The listing builds one solid part. Answer for the finished solid, in the listing's coordinates (mm). Face numbers are marked on the shaded views. A direction names the side the tool comes from. Round coordinates to 2 decimals unless told otherwise and drop trailing zeros. Order: outer loops, then holes, each group sorted by start corner. A loop starts at its lowest first (then second) coordinate and runs counter-clockwise, first axis right, second up. Notation, with made-up numbers: M 46,52 L 89,52 A24 ccw 89,77 Z; hole C 10,-18 d6. An arc over 180 degrees is marked long. Put each result on its own line as item: value. Start each with the question number.
1. The part is cut by section C-C (y = 59.5). Give the vertices of the cut face in (x, z), then the cut area to 3 significant figures.
2. The part is cut by section A-A (z = 10). Count the separate pieces of the cut face and the enclosed holes in it, then the cut area to 3 significant figures.
3. The part is cut by section D-D (z = -8.5). Give the vertices of the cut face in (x, y), then the cut area to 3 significant figures.
4. Each of these flat-tipped pins is pushed along its axis until it touches: pin 1 Ø6 at (x, z) = (0, -4.5) entering from -Y; pin 2 Ø3 at (x, y) = (20.5, 45.5) entering from +Z; pin 3 Ø4 at (y, z) = (50, 13.5) entering from -X. Where does it stop, or does it pass through?
5. Which of the six approach directions +Z, -Z, +X, -X, +Y, -Y give full straight-line access (tool end or side, diameter ignored) to the marked faces 5, 6 and 7?
6. Consider line 1 (X direction, y = 57.75, z = 10); line 2 (Y direction, x = -5, z = -6.5); line 3 (Y direction, x = 6, z = 39.5). Determine where each line is inside the solid, lowest interval first.
7. The mould has two halves that part along Y. Classify the marked faces 1, 2, 3 and 4: +Y half, -Y half, draft (parallel to the pull), parting line (faces both ways), or undercut.
8. The part is cut by section B-B (x = 9). Give the vertices of the cut face in (y, z), then the cut area to 3 significant figures.
from build123d import *

# Parameters (mm, degrees)
BOSS_EXTRUDE4_DEPTH      = 20
BOSS_EXTRUDE5_REACH      = 41.361
BOSS_EXTRUDE5_END_RADIUS = 37.5
SKETCH8_R                = 10
SKETCH9_R                = 20
BOSS_EXTRUDE6_DEPTH      = 5
SKETCH10_R               = 32.5
BOSS_EXTRUDE7_DEPTH      = 20
SKETCH11_R               = 20
BOSS_EXTRUDE8_DEPTH      = 5
SKETCH12_R               = 10
CUT_EXTRUDE3_DEPTH       = 20


with BuildPart() as part:
    # Sketch4 → Boss-Extrude4 (new body)
    with BuildSketch(Plane.XY):
        with BuildLine():
            Line((-26.811555509, 22.497566339), (-28.726666617, 24.104535363))
            ThreePointArc((-28.726666617, 24.104535363), (0, 37.5), (28.726666617, 24.104535363))
            Line((28.726666617, 24.104535363), (26.811555509, 22.497566339))
            ThreePointArc((26.811555509, 22.497566339), (0, 35), (-26.811555509, 22.497566339))
        make_face()
    extrude(amount=BOSS_EXTRUDE4_DEPTH)

    # Boss-Extrude5: up to this cylinder (the profile starts outside it)
    boss_extrude5_end = Plane(origin=(0, 0, 10), z_dir=(0, 0, -1)) * Cylinder(BOSS_EXTRUDE5_END_RADIUS, 158.722, mode=Mode.PRIVATE)
    # Sketch8 → Boss-Extrude5 (add, up to the surface)
    with BuildSketch(Plane(origin=(0, 40.5, 0), x_dir=(1, 0, 0), z_dir=(0, 1, 0)), mode=Mode.PRIVATE) as boss_extrude5_sk1:
        with Locations(Location((0, -10, 0), (0, 0, 270))):
            Circle(SKETCH8_R)
    boss_extrude5_tool1 = extrude(boss_extrude5_sk1.sketch, amount=-BOSS_EXTRUDE5_REACH, mode=Mode.PRIVATE) - boss_extrude5_end
    add(boss_extrude5_tool1.solids().sort_by_distance((0, 40.5, 10))[0])

    # Sketch9 → Boss-Extrude6 (add)
    with BuildSketch(Plane(origin=(0, 40.5, 0), x_dir=(1, 0, 0), z_dir=(0, 1, 0))):
        with Locations(Location((0, -10, 0), (0, 0, 270))):
            Circle(SKETCH9_R)
    extrude(amount=BOSS_EXTRUDE6_DEPTH)

    # Sketch10 → Boss-Extrude7 (add)
    with BuildSketch(Plane(origin=(0, 45.5, 0), x_dir=(1, 0, 0), z_dir=(0, 1, 0))):
        with Locations(Location((0, -10, 0), (0, 0, 270))):
            Circle(SKETCH10_R)
    extrude(amount=BOSS_EXTRUDE7_DEPTH)

    # Sketch11 → Boss-Extrude8 (add)
    with BuildSketch(Plane(origin=(0, 65.5, 0), x_dir=(1, 0, 0), z_dir=(0, 1, 0))):
        with Locations(Location((0, -10, 0), (0, 0, 270))):
            Circle(SKETCH11_R)
    extrude(amount=BOSS_EXTRUDE8_DEPTH)

    # Sketch12 → Cut-Extrude3 (cut)
    with BuildSketch(Plane(origin=(0, 70.5, 0), x_dir=(1, 0, 0), z_dir=(0, 1, 0))):
        with Locations(Location((0, -10, 0), (0, 0, 270))):
            Circle(SKETCH12_R)
    extrude(amount=-CUT_EXTRUDE3_DEPTH, mode=Mode.SUBTRACT)

    # Sketch15 → Cut-Revolve3 (revolve, cut)
    with BuildSketch(Plane.XY.offset(10), mode=Mode.PRIVATE) as cut_revolve3_sk:
        Polygon((-17.693131792, 21.085853377), (-26.278152948, 31.317083182), (-30.108375164, 28.103145134), (-21.523354007, 17.871915328), align=None)
    revolve(cut_revolve3_sk.sketch.rotate(Axis((-17.693131792, 21.085853377, 10), (-0.6427876096865413, 0.7660444431189765, 0)), 180), axis=Axis((-17.693131792, 21.085853377, 10), (-0.6427876096865413, 0.7660444431189765, 0)), mode=Mode.SUBTRACT)

    # Sketch16 → Cut-Revolve4 (revolve, cut)
    with BuildSketch(Plane.XY.offset(10), mode=Mode.PRIVATE) as cut_revolve4_sk:
        Polygon((17.792638641, 21.204441023), (27.637153268, 32.936676696), (23.806931052, 36.150614744), (13.962416426, 24.418379071), align=None)
    revolve(cut_revolve4_sk.sketch.rotate(Axis((17.792638641, 21.204441023, 10), (0.6427876096865399, 0.7660444431189776, 0)), 180), axis=Axis((17.792638641, 21.204441023, 10), (0.6427876096865399, 0.7660444431189776, 0)), mode=Mode.SUBTRACT)


solid = part.part
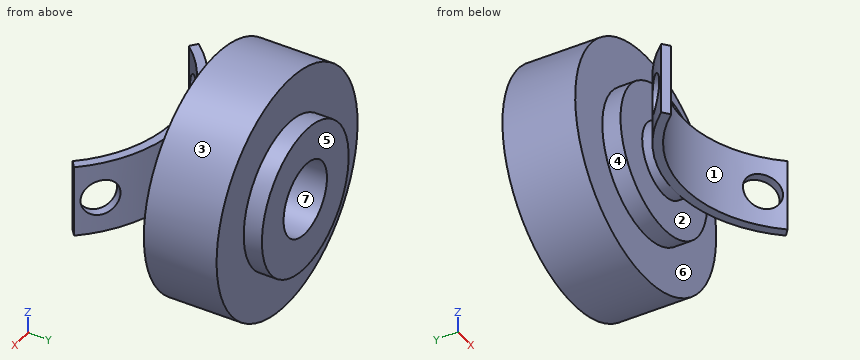
Resolved:
1. outline: C 0,10 d65; hole C 0,10 d20
1. area: 3,000 mm2
2. separate pieces: 3
2. enclosed holes: 0
2. area: 1,480 mm2
3. outline: M -26.72,45.5 L -7.6,45.5 L -7.6,40.5 L 7.6,40.5 L 7.6,45.5 L 26.72,45.5 L 26.72,65.5 L 7.6,65.5 L 7.6,70.5 L -7.6,70.5 L -7.6,65.5 L -26.72,65.5 Z
3. area: 1,220 mm2
4. pin 1: y = 40.5
4. pin 2: z = 36.37
4. pin 3: x = -32.47
5. face 5: +Z, -Z, +X, -X, +Y
5. face 6: none
5. face 7: +Y
6. line 1: -32.5 to -10, 10 to 32.5
6. line 2: 40.5 to 70.5
6. line 3: 45.5 to 65.5
7. face 1: -Y half
7. face 2: undercut
7. face 3: draft
7. face 4: undercut
8. outline: M 33.82,0 L 36.4,0 L 36.4,5.64 L 40.5,5.64 L 40.5,-7.86 L 45.5,-7.86 L 45.5,-21.23 L 65.5,-21.23 L 65.5,-7.86 L 70.5,-7.86 L 70.5,5.64 L 50.5,5.64 L 50.5,14.36 L 70.5,14.36 L 70.5,27.86 L 65.5,27.86 L 65.5,41.23 L 45.5,41.23 L 45.5,27.86 L 40.5,27.86 L 40.5,14.36 L 36.4,14.36 L 36.4,20 L 33.82,20 Z
8. area: 1,520 mm2
